```python
from build123d import *

# Parameters (mm, degrees)
SKETCH_1_R              = 45
EXTRUDE_1_DEPTH         = 12
SKETCH_2_R              = 30
EXTRUDE_2_DEPTH         = 50
SKETCH_11_R             = 34
EXTRUDE_3_DEPTH         = 3
SKETCH_3_R              = 23
CUT_EXTRUDE_1_DEPTH     = 89.848185125
CHAMFER_1_SIZE          = 1
HOLE_WIZARD_M5_1_D      = 4.2
CUT_EXTRUDE_2_DEPTH     = 89.848185125
HOLE_WIZARD_M8_1_REACH  = 118.675
HOLE_WIZARD_M8_1_BORE_R = 3.4


with BuildPart() as part:
    # 草图1 → 凸台-拉伸1 (new body)
    with BuildSketch(Plane(origin=(0, 0, 0), x_dir=(1, 0, 0), z_dir=(0, 1, 0))):
        with Locations(Location((0, 0, 0), (0, 0, 270))):
            Circle(SKETCH_1_R)
    extrude(amount=EXTRUDE_1_DEPTH)

    # 草图2 → 凸台-拉伸2 (add)
    with BuildSketch(Plane(origin=(0, 12, 0), x_dir=(1, 0, 0), z_dir=(0, 1, 0))):
        with Locations(Location((0, 0, 0), (0, 0, 270))):
            Circle(SKETCH_2_R)
    extrude(amount=EXTRUDE_2_DEPTH)

    # 草图11 → 凸台-拉伸3 (add)
    with BuildSketch(Plane(origin=(0, 12, 0), x_dir=(1, 0, 0), z_dir=(0, 1, 0))):
        with Locations(Location((0, 0, 0), (0, 0, 270))):
            Circle(SKETCH_11_R)
    extrude(amount=EXTRUDE_3_DEPTH)

    # 草图3 → 切除-拉伸1 (cut, through all)
    with BuildSketch(Plane.XZ):
        with Locations(Location((0, 0, 0), (0, 0, 270))):
            Circle(SKETCH_3_R)
    extrude(amount=-CUT_EXTRUDE_1_DEPTH, mode=Mode.SUBTRACT)

    # 倒角1
    chamfer_1_edges = [part.edges().sort_by_distance(p)[0] for p in [
        (0, 15, -34),
        (0, 62, 23),
        (0, 0, 23),
        (0, 0, -45),
        (0, 12, -45),
        (0, 62, -30),
    ]]
    chamfer(chamfer_1_edges, length=CHAMFER_1_SIZE)

    # M5 螺纹孔1 (through all)
    with Locations(Plane(origin=(0, 0, 0), x_dir=(-1, 0, 0), z_dir=(0, -1, 0))):
        with Locations((25, -25), (-25, -25), (-25, 25), (25, 25)):
            Hole(HOLE_WIZARD_M5_1_D / 2)

    # 草图8 → 切除-拉伸2 (cut, through all)
    with BuildSketch(Plane.XZ):
        with BuildLine():
            Line((-13.266499161, 43), (13.266499161, 43))
            ThreePointArc((13.266499161, 43), (0, 45), (-13.266499161, 43))
        make_face()
    extrude(amount=-CUT_EXTRUDE_2_DEPTH, mode=Mode.SUBTRACT)

    # M8 螺纹孔1 bore → M8 螺纹孔1 (cut, up to next)
    with BuildSketch(Plane.XY.offset(43), mode=Mode.PRIVATE) as hole_wizard_m8_1_sk1:
        with Locations((0, 6)):
            Circle(HOLE_WIZARD_M8_1_BORE_R)
    hole_wizard_m8_1_tool1 = extrude(hole_wizard_m8_1_sk1.sketch, amount=-HOLE_WIZARD_M8_1_REACH, mode=Mode.PRIVATE) & part.part
    add(hole_wizard_m8_1_tool1.solids().sort_by_distance((0, 6, 43))[0], mode=Mode.SUBTRACT)


solid = part.part
```
Verification items for the finished model (mm, model axes). A direction names the side the tool comes from. Round coordinates to 2 decimals unless told otherwise and drop trailing zeros. Order: outer loops, then holes, each group sorted by start corner. A loop starts at its lowest first (then second) coordinate and runs counter-clockwise, first axis right, second up.
1) Cross-section at A-A, the plane z = 0. Record the cut outline in (x, y).
Geometry says:
outline: (-45, 1) - (-44, 0) - (-24, 0) - (-23, 1) - (-23, 61) - (-24, 62) - (-29, 62) - (-30, 61) - (-30, 15) - (-33, 15) - (-34, 14) - (-34, 12) - (-44, 12) - (-45, 11) - close; (23, 1) - (24, 0) - (44, 0) - (45, 1) - (45, 11) - (44, 12) - (34, 12) - (34, 14) - (33, 15) - (30, 15) - (30, 61) - (29, 62) - (24, 62) - (23, 61) - close
2) Tool access check on faces 1 (the cylindrical face through (0, 13, -34)), 2 (the cylindrical face through (-34, 13, 0)), 3 (the cylindrical face through (1.32, 37.68, -29.97)), 4 (the cylindrical face through (34, 13, 0)). Record the directions out of +Z, -Z, +X, -X, +Y, -Y that give a thin tool (end or side, any length) a straight path to the whole face; none if there is none.
Geometry says:
face 1: -Z, +Y
face 2: -X, +Y
face 3: +Y
face 4: +X, +Y
3) Cross-section at C-C, the plane y = 6. Record the cut outline in (x, z), plus the area to 3 significant figures.
Geometry says:
outline: (-13.27, 43) arc R45 ccw (long way) to (13.27, 43) - (3.4, 43) - (3.4, 22.75) arc R23 cw (long way) to (-3.4, 22.75) - (-3.4, 43) - close; hole circle Ø4.2 at (-25, -25); hole circle Ø4.2 at (-25, 25); hole circle Ø4.2 at (25, -25); hole circle Ø4.2 at (25, 25)
area: 4,470 mm2
4) Depth check by flat-ended pin: pin 1 (3 mm diameter, centred on x = 0, y = 50, fed in from +Z); pin 2 (6 mm diameter, centred on y = 39.5, z = 28.5, fed in from +X); pin 3 (20 mm diameter, centred on x = 7.5, z = -13.5, fed in from +Y); pin 4 (5.5 mm diameter, centred on x = 25, z = -25, fed in from +Y). Enter the tip coordinate at first touch or a pass-through.
Geometry says:
pin 1: stops at z = 30
pin 2: stops at x = 15.8
pin 3: stops at y = 62
pin 4: stops at y = 15
5) Material ranges on line 1 (Z direction, x = -25, y = 10); line 2 (X direction, y = 10, z = 0.5); line 3 (X direction, y = 9, z = 25), recorded low to high.
Geometry says:
line 1: z = -37.42 to -27.1, -22.9 to 22.9, 27.1 to 37.42
line 2: x = -45 to -22.99, 22.99 to 45
line 3: x = -37.42 to -27.1, -22.9 to -1.6, 1.6 to 22.9, 27.1 to 37.42
6) Cross-section at D-D, the plane y = 52. Record the cut outline in (x, z), plus the area to 3 significant figures.
Geometry says:
outline: circle Ø60 at (0, 0); hole circle Ø46 at (0, 0)
area: 1,170 mm2
7) Draft check along Y on faces 5 (the cylindrical face through (-0.44, 9.37, 33.02)), 6 (the conical face through (1.81, 0.16, -44.123)), 7 (the flat face through (-27, 15, 15)), 8 (the cylindrical face through (23.334, 5.837, -23.722)). Enter one of: +Y half, -Y half, draft (parallel to the pull), parting line (faces both ways), or undercut.
Geometry says:
face 5: undercut
face 6: -Y half
face 7: +Y half
face 8: draft
8) Cross-section at B-B, the plane x = 0. Give the number of separate pieces and of enclosed holes in the cut face, plus the area to 3 significant figures.
Geometry says:
separate pieces: 3
enclosed holes: 0
area: 1,090 mm2
